Check sheet for the drawn part. Datum: minimum x, y, z corner. Units: mm. Give positions to 0.01 mm unless a question says otherwise; leave off trailing zeros. Loops run counter-clockwise (first coordinate to the right, second up) from the corner with the lowest first, then second, coordinate; pieces in that order, holes last.
1. Cross-section at A-A, the plane x = 10. Record the cut outline in (y, z), plus the area to 3 significant figures.
2. Go/stop test with a flat-tipped pin: pin 1 Ø4 at (x, z) = (10, 115) entering from -Y. Record where the tip stops, or that it passes through.
3. Cross-section at C-C, the plane z = 115. Record the cut outline in (x, y), plus the area to 3 significant figures.
4. Material ranges on L1, parallel to Z at x = 10, y = 16.75; L2, parallel to X at y = 12, z = 115; L3, parallel to Z at x = 9, y = 8, recorded low to high.
5. Cross-section at B-B, the plane y = 17. Record the cut outline in (x, z), plus the area to 3 significant figures.
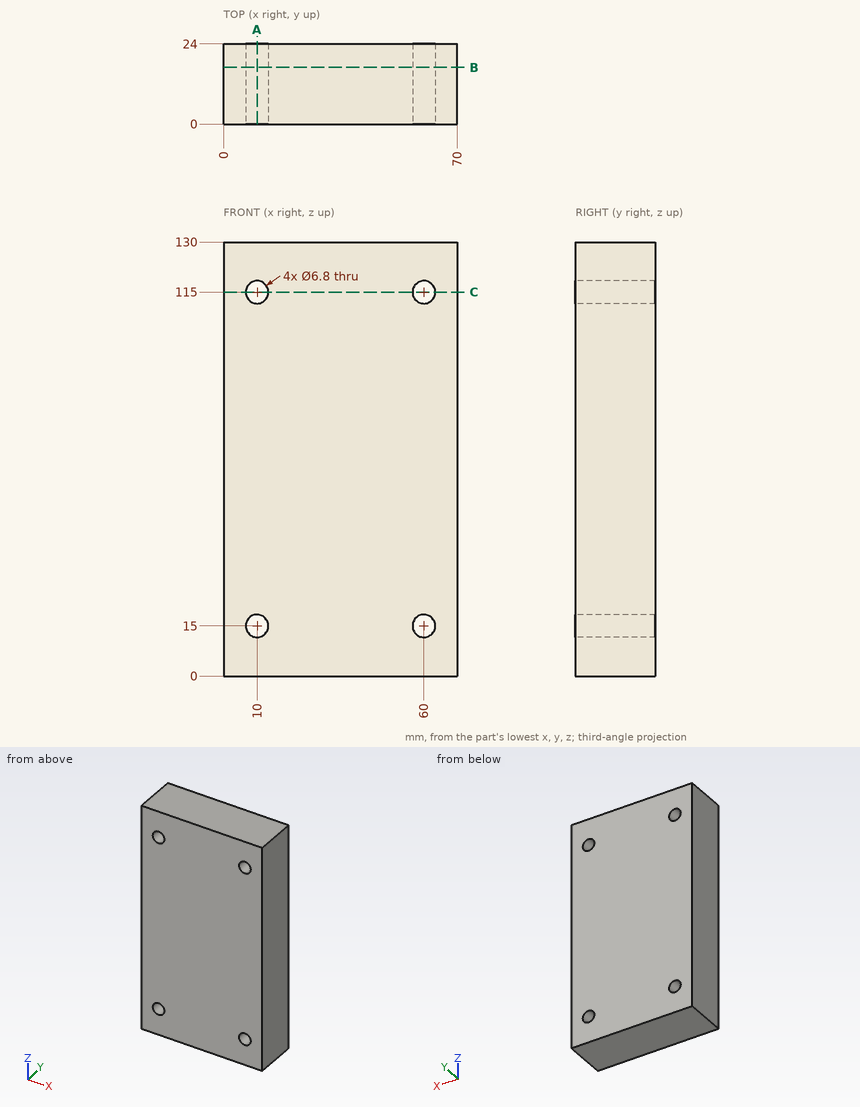
Result:
1. outline: (0, 0) - (24, 0) - (24, 11.6) - (0, 11.6) - close; (0, 18.4) - (24, 18.4) - (24, 111.6) - (0, 111.6) - close; (0, 118.4) - (24, 118.4) - (24, 130) - (0, 130) - close
1. area: 2,790 mm2
2. pin 1: passes through
3. outline: (0, 0) - (6.6, 0) - (6.6, 24) - (0, 24) - close; (13.4, 0) - (56.6, 0) - (56.6, 24) - (13.4, 24) - close; (63.4, 0) - (70, 0) - (70, 24) - (63.4, 24) - close
3. area: 1,350 mm2
4. L1: z = 0 to 11.6, 18.4 to 111.6, 118.4 to 130
4. L2: x = 0 to 6.6, 13.4 to 56.6, 63.4 to 70
4. L3: z = 0 to 11.75, 18.25 to 111.75, 118.25 to 130
5. outline: (0, 0) - (70, 0) - (70, 130) - (0, 130) - close; hole circle Ø6.8 at (10, 15); hole circle Ø6.8 at (10, 115); hole circle Ø6.8 at (60, 15); hole circle Ø6.8 at (60, 115)
5. area: 8,950 mm2
